Input: part model. Units: mm. Frame: model coordinates. A direction names the side the tool comes from. Round coordinates to 2 decimals unless told otherwise and drop trailing zeros. Order: outer loops, then holes, each group sorted by start corner. A loop starts at its lowest first (then second) coordinate and runs counter-clockwise, first axis right, second up. Notation, with made-up numbers: (24.5, -17.75) -> (37.5, -17.75) arc R10 ccw to (37.5, -12.75) -> close; hole circle Ø7 at (-22, 44). An arc over 180 degrees is marked (long way). Answer as CSV lines item,"result". Start each with the question number.
1) Section query A-A, the plane y = 341.5. Output: boundary loops of the cut face in (x, z), and give its area (3 significant figures).
2) Line query: L1, parallel to Y at x = 47, z = 7; L2, parallel to X at y = 0.9, z = 12; L3, parallel to X at y = 1.25, z = -42. Output: solid intervals per line, ascending.
3) Access query for faces 1 (the face through (116.985, 1254.986, -43.407)), 2 (the face through (26, 619, 0)), 3 (the face through (93, 2, -23)), 4 (the face through (27, 619, 2)). Directions: +Z, -Z, +X, -X, +Y, -Y. A direction counts if a zero-diameter tool reaches every point of the face in a straight line with its end or side. Return the directions, or none.
4) Section query D-D, the plane z = -64. Output: boundary loops of the cut face in (x, y), and give its area (3 significant figures).
5) Section query B-B, the plane x = 39. Output: boundary loops of the cut face in (y, z), and give its area (3 significant figures).
6) Mould query, pull axis Y, two halves, no side actions, for faces 5 (the face through (94.667, 619.236, -27.864)), 6 (the face through (89, 0, -19)), 7 (the face through (0, 625.1, 0.5)). Classes: +Y half, -Y half, draft (parallel to the pull), parting line (faces both ways), or undercut.
7) Section query C-C, the plane y = 565. Output: boundary loops of the cut face in (x, z).
8) First-contact query: P1, Ø3, axis at x = 12, y = 493.5, coming from the -Z side; P2, Ø3, axis at x = 71, y = 726.5, coming from the +Z side; P3, Ø3, axis at x = 17, y = 596, coming from the +Z side; P4, Ø1.5, axis at y = 1104, z = -88, coming from the -X side. Flat tips, straight axial feed; report the tip coordinate or a pass-through.
```python
from build123d import *

# Parameters (mm, degrees)
EXTRUDE_1_DEPTH     = 1256
EXTRUDE_START       = -2
EXTRUDE_2_DEPTH     = 2
EXTRUDE_3_DEPTH     = 2
SKETCH_5_W          = 15
SKETCH_5_H          = 100
CUT_EXTRUDE_2_DEPTH = 265
SKETCH_6_R          = 2.75
CUT_EXTRUDE_3_DEPTH = 1510


with BuildPart() as part:
    # 草图1 → 凸台-拉伸1 (new body)
    with BuildSketch(Plane(origin=(0, 0, 0), x_dir=(1, 0, 0), z_dir=(0, 1, 0))):
        with BuildLine():
            Line((0, 0), (53, 0))
            ThreePointArc((53, 0), (95, 42), (53, 84))
            Line((53, 84), (53, 86))
            ThreePointArc((53, 86), (97, 42), (53, -2))
            Line((53, -2), (0, -2))
            Line((0, -2), (0, 0))
        make_face()
    extrude(amount=EXTRUDE_1_DEPTH)

    # 草图3 → 凸台-拉伸2 (add)
    with BuildSketch(Plane(origin=(0, 1256, 0), x_dir=(1, 0, 0), z_dir=(0, 1, 0)).offset(EXTRUDE_START)):
        with BuildLine():
            Line((0, 0), (53, 0))
            ThreePointArc((53, 0), (95, 42), (53, 84))
            Line((53, 84), (53, 106))
            ThreePointArc((53, 106), (117, 42), (53, -22))
            Line((53, -22), (0, -22))
            Line((0, -22), (0, 0))
        make_face()
    extrude(amount=EXTRUDE_2_DEPTH)

    # 草图4 → 凸台-拉伸3 (add)
    with BuildSketch(Plane.XZ):
        with BuildLine():
            Line((53, 0), (0, 0))
            Line((0, 0), (0, 2))
            Line((0, 2), (0, 22))
            Line((0, 22), (53, 22))
            ThreePointArc((53, 22), (117, -42), (53, -106))
            Line((53, -106), (53, -86))
            Line((53, -86), (53, -84))
            ThreePointArc((53, -84), (95, -42), (53, 0))
        make_face()
    extrude(amount=-EXTRUDE_3_DEPTH)

    # 草图5 → 切除-拉伸2 (cut)
    with BuildSketch(Plane(origin=(0, 0, 0), x_dir=(0, 0, -1), z_dir=(1, 0, 0))):
        with Locations((42.25, 65.421277154)):
            Rectangle(SKETCH_5_W, SKETCH_5_H)
        with Locations((42.25, 208)):
            Rectangle(SKETCH_5_W, SKETCH_5_H)
        with Locations((42.25, 1048)):
            Rectangle(SKETCH_5_W, SKETCH_5_H)
        with Locations((42.25, 348)):
            Rectangle(SKETCH_5_W, SKETCH_5_H)
        with Locations((42.25, 488)):
            Rectangle(SKETCH_5_W, SKETCH_5_H)
        with Locations((42.25, 628)):
            Rectangle(SKETCH_5_W, SKETCH_5_H)
        with Locations((42.25, 768)):
            Rectangle(SKETCH_5_W, SKETCH_5_H)
        with Locations((42.25, 908)):
            Rectangle(SKETCH_5_W, SKETCH_5_H)
        with Locations((42.25, 1188)):
            Rectangle(SKETCH_5_W, SKETCH_5_H)
    extrude(amount=CUT_EXTRUDE_2_DEPTH, mode=Mode.SUBTRACT)

    # 草图6 → 切除-拉伸3 (cut)
    with BuildSketch(Plane(origin=(0, 1256, 0), x_dir=(1, 0, 0), z_dir=(0, 1, 0))):
        with Locations(Location((80, 88.765371804, 0), (0, 0, 270))):
            Circle(SKETCH_6_R)
        with Locations(Location((107, 42, 0), (0, 0, 270))):
            Circle(SKETCH_6_R)
        with Locations(Location((53, -12, 0), (0, 0, 270))):
            Circle(SKETCH_6_R)
        with Locations(Location((8, -12, 0), (0, 0, 270))):
            Circle(SKETCH_6_R)
    extrude(amount=-CUT_EXTRUDE_3_DEPTH, mode=Mode.SUBTRACT)


solid = part.part
```
Findings:
1,outline,"(0, 0) -> (53, 0) arc R42 cw to (94.37, -34.75) -> (96.4, -34.75) arc R44 ccw to (53, 2) -> (0, 2) -> close; (53, -86) arc R44 ccw to (96.31, -49.75) -> (94.28, -49.75) arc R42 cw to (53, -84) -> close"
1,area,"346 mm^2"
2,L1,"y = 0 to 2, 1254 to 1256"
2,L2,"x = 0 to 5.25, 10.75 to 50.25, 55.75 to 87.35"
2,L3,"x = 95 to 104.25, 109.75 to 117"
3,face 1,"+X, +Y, -Y"
3,face 2,"-Z, -X, +Y, -Y"
3,face 3,"+X"
3,face 4,"+Z, +X, -X"
4,outline,"(88.78, 0) -> (113.1, 0) -> (113.1, 2) -> (91.11, 2) -> (91.11, 1254) -> (113.1, 1254) -> (113.1, 1256) -> (88.78, 1256) -> close"
4,area,"3,010 mm^2"
5,outline,"(0, 0) -> (1256, 0) -> (1256, 22) -> (1254, 22) -> (1254, 2) -> (2, 2) -> (2, 22) -> (0, 22) -> close"
5,area,"2,590 mm^2"
6,face 5,"undercut"
6,face 6,"-Y half"
6,face 7,"draft"
7,outline,"(0, 0) -> (53, 0) arc R42 cw to (53, -84) -> (53, -86) arc R44 ccw to (53, 2) -> (0, 2) -> close"
8,P1,"stops at z = 0"
8,P2,"stops at z = -1.21"
8,P3,"stops at z = 2"
8,P4,"passes through"
